Design review of the part built by this model. Coordinates are the model's own, in mm. Face numbers are marked on the shaded views. Coordinates: 2 decimals unless noted, no trailing zeros. Write each loop counter-clockwise with the first axis right and the second up, starting at its lowest first coordinate (ties: lowest second). Pieces come first, ordered by that corner, then holes. Notation, with made-up numbers: (53, 0) - (91, 0) arc R14 cw to (91, 14) - close; hole circle Ø5 at (48.5, 15). An arc over 180 degrees is marked (long way). Use a Markdown table: item, result.
from build123d import *

# Parameters (mm, degrees)
SKETCH1_R             = 40
SKETCH1_R_2           = 30
BOSS_EXTRUDE1_DEPTH   = 864.5
SKETCH2_OUTSIDE_W     = 256.374
SKETCH2_OUTSIDE_H     = 256.374
SKETCH2_OUTSIDE_R     = 37.5
CUT_EXTRUDE1_DEPTH    = 25
SKETCH3_OUTSIDE_W     = 256.374
SKETCH3_OUTSIDE_H     = 256.374
SKETCH3_OUTSIDE_R     = 36.5
CUT_EXTRUDE2_DEPTH    = 3
SKETCH4_OUTSIDE_W     = 256.374
SKETCH4_OUTSIDE_H     = 256.374
SKETCH4_OUTSIDE_R     = 38
CUT_EXTRUDE3_DEPTH    = 2
SKETCH5_R             = 32.5
CUT_EXTRUDE4_DEPTH    = 50
CHAMFER2_SIZE         = 1.5
M5_TAPPED_HOLE1_D     = 4.2
M5_TAPPED_HOLE1_DEPTH = 10
M5_TAPPED_HOLE1_TIP   = 1.2618073
SKETCH8_R             = 4
CUT_EXTRUDE5_DEPTH    = 30


with BuildPart() as part:
    # Sketch1 → Boss-Extrude1 (new body)
    with BuildSketch(Plane(origin=(0, 0, 0), x_dir=(1, 0, 0), z_dir=(0, 1, 0))):
        with Locations(Location((0, 0, 0), (0, 0, 270))):
            Circle(SKETCH1_R)
        with Locations(Location((0, 0, 0), (0, 0, 270))):
            Circle(SKETCH1_R_2, mode=Mode.SUBTRACT)
    extrude(amount=BOSS_EXTRUDE1_DEPTH)

    # Sketch2 outside → Cut-Extrude1 (cut)
    with BuildSketch(Plane(origin=(0, 864.5, 0), x_dir=(1, 0, 0), z_dir=(0, 1, 0))):
        Rectangle(SKETCH2_OUTSIDE_W, SKETCH2_OUTSIDE_H)
        with Locations(Location((0, 0, 0), (0, 0, 270))):
            Circle(SKETCH2_OUTSIDE_R, mode=Mode.SUBTRACT)
    extrude(amount=-CUT_EXTRUDE1_DEPTH, mode=Mode.SUBTRACT)

    # Sketch3 outside → Cut-Extrude2 (cut)
    with BuildSketch(Plane(origin=(0, 839.5, 0), x_dir=(1, 0, 0), z_dir=(0, 1, 0))):
        Rectangle(SKETCH3_OUTSIDE_W, SKETCH3_OUTSIDE_H)
        with Locations(Location((0, 0, 0), (0, 0, 270))):
            Circle(SKETCH3_OUTSIDE_R, mode=Mode.SUBTRACT)
    extrude(amount=-CUT_EXTRUDE2_DEPTH, mode=Mode.SUBTRACT)

    # Sketch4 outside → Cut-Extrude3 (cut)
    with BuildSketch(Plane(origin=(0, 836.5, 0), x_dir=(1, 0, 0), z_dir=(0, 1, 0))):
        Rectangle(SKETCH4_OUTSIDE_W, SKETCH4_OUTSIDE_H)
        with Locations(Location((0, 0, 0), (0, 0, 270))):
            Circle(SKETCH4_OUTSIDE_R, mode=Mode.SUBTRACT)
    extrude(amount=-CUT_EXTRUDE3_DEPTH, mode=Mode.SUBTRACT)

    # Sketch5 → Cut-Extrude4 (cut)
    with BuildSketch(Plane.XZ):
        with Locations(Location((0, 0, 0), (0, 0, 270))):
            Circle(SKETCH5_R)
    extrude(amount=-CUT_EXTRUDE4_DEPTH, mode=Mode.SUBTRACT)

    # Chamfer2
    chamfer2_edges = [part.edges().sort_by_distance(p)[0] for p in [
        (0, 50, -30),
    ]]
    chamfer(chamfer2_edges, length=CHAMFER2_SIZE)

    # M5 Tapped Hole1
    with Locations(Plane.XY.offset(40)):
        with Locations((0, 9)):
            Hole(M5_TAPPED_HOLE1_D / 2, depth=M5_TAPPED_HOLE1_DEPTH)
            with Locations((0, 0, -(M5_TAPPED_HOLE1_DEPTH + M5_TAPPED_HOLE1_TIP / 2))):  # 118° drill point
                Cone(0, M5_TAPPED_HOLE1_D / 2, M5_TAPPED_HOLE1_TIP, mode=Mode.SUBTRACT)

    # Sketch8 → Cut-Extrude5 (cut)
    with BuildSketch(Plane.XY.offset(40)):
        with Locations((0, 819.5)):
            Circle(SKETCH8_R)
    extrude(amount=-CUT_EXTRUDE5_DEPTH, mode=Mode.SUBTRACT)


solid = part.part
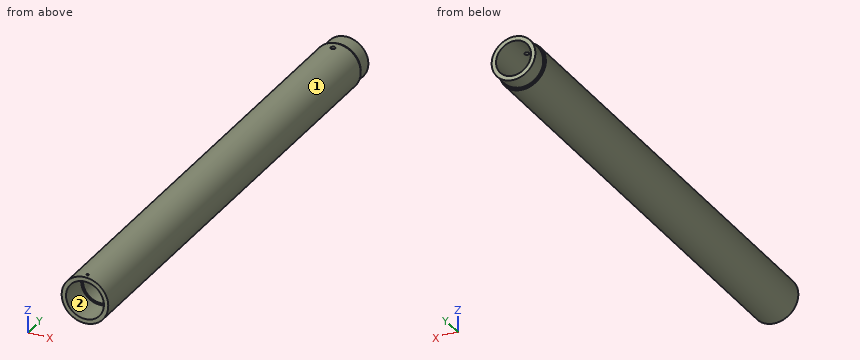
(1) Take a section at A-A on z = 0. Write out the cut boundary in (x, y).
Determined:
| item | result |
|---|---|
| outline | (-40, 0) - (-32.5, 0) - (-32.5, 50) - (-31.5, 50) - (-30, 51.5) - (-30, 864.5) - (-37.5, 864.5) - (-37.5, 839.5) - (-36.5, 839.5) - (-36.5, 836.5) - (-38, 836.5) - (-38, 834.5) - (-40, 834.5) - close; (30, 51.5) - (31.5, 50) - (32.5, 50) - (32.5, 0) - (40, 0) - (40, 834.5) - (38, 834.5) - (38, 836.5) - (36.5, 836.5) - (36.5, 839.5) - (37.5, 839.5) - (37.5, 864.5) - (30, 864.5) - close |
(2) For pin 1 (3.5 mm diameter, centred on x = 0, y = 9, fed in from +Z); pin 2 (2 mm diameter, centred on x = -9, y = 541, fed in from -Z); pin 3 (6 mm diameter, centred on x = 18.5, y = 283, fed in from +Z), all flat-tipped, find the tip position at first contact; note any pin that passes through.
Determined:
| item | result |
|---|---|
| pin 1 | z = -32.45 |
| pin 2 | z = -39.19 |
| pin 3 | z = 36.87 |
(3) Take a section at B-B on y = 585. Write out the cut boundary in (x, z).
Determined:
| item | result |
|---|---|
| outline | circle Ø80 at (0, 0); hole circle Ø60 at (0, 0) |
(4) Draft analysis for pull direction X (two halves, no side actions). For the marked faces 1 and 2, state which applies: +X half, -X half, draft (parallel to the pull), parting line (faces both ways), or undercut.
Determined:
| item | result |
|---|---|
| face 1 | parting line |
| face 2 | undercut |
(5) For L1, parallel to Y at x = 0, z = 33; L2, parallel to Z at x = 0, y = 34.5; L3, parallel to X at y = 553, z = 0, list the stretches that pass through material, from the lowest coordinate up. Write a range as from..to.
Determined:
| item | result |
|---|---|
| L1 | 0..6.9, 11.1..815.5, 823.5..864.5 |
| L2 | -40..-32.5, 32.5..40 |
| L3 | -40..-30, 30..40 |
